Geometry check sheet. Reference: the model listing, model coordinates, mm. Face numbers are marked on the shaded views. A direction names the side the tool comes from. Round coordinates to 2 decimals unless told otherwise and drop trailing zeros. Write each loop counter-clockwise with the first axis right and the second up, starting at its lowest first coordinate (ties: lowest second). Pieces come first, ordered by that corner, then holes. Notation, with made-up numbers: (34.25, -5) -> (62.25, -5) arc R13 cw to (62.25, 18) -> close; hole circle Ø2 at (-36, 0.25). An arc over 180 degrees is marked (long way). Put each result on its own line as item: value. Start each with the question number.
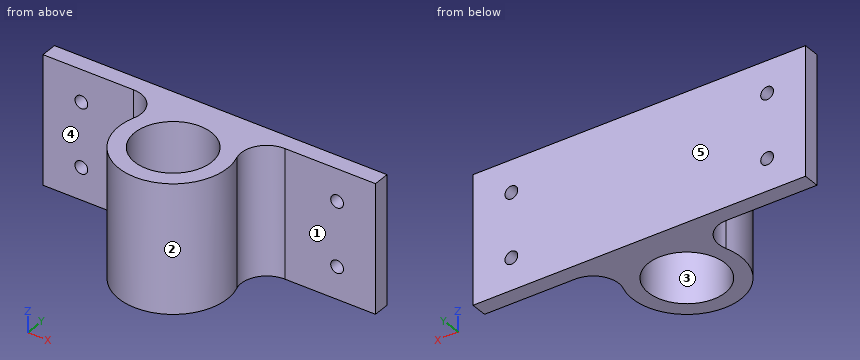
from build123d import *

# Parameters (mm, degrees)
SKETCH1_R           = 75
BOSS_EXTRUDE1_DEPTH = 250
CUT_EXTRUDE1_REACH  = 476.098
SKETCH2_R           = 12.5


with BuildPart() as part:
    # Sketch1 → Boss-Extrude1 (new body)
    with BuildSketch(Plane.XY):
        with BuildLine():
            Line((325, 132), (-325, 132))
            Line((-325, 132), (-325, 100))
            Line((-325, 100), (-147.770091697, 100))
            ThreePointArc((-147.770091697, 100), (-107.142009959, 79.143763902), (-100.407882819, 33.974358974))
            ThreePointArc((-100.407882819, 33.974358974), (0, -106), (100.407882819, 33.974358974))
            ThreePointArc((100.407882819, 33.974358974), (107.142009959, 79.143763902), (147.770091697, 100))
            Line((147.770091697, 100), (325, 100))
            Line((325, 100), (325, 132))
        make_face()
        Circle(SKETCH1_R, mode=Mode.SUBTRACT)
    extrude(amount=BOSS_EXTRUDE1_DEPTH)

    # Sketch2 → Cut-Extrude1 (cut, up to next)
    with BuildSketch(Plane(origin=(0, 132, 0), x_dir=(1, 0, 0), z_dir=(0, 1, 0)), mode=Mode.PRIVATE) as cut_extrude1_sk1:
        with Locations(Location((-250, -62.5, 0), (0, 0, 270))):
            Circle(SKETCH2_R)
    cut_extrude1_tool1 = extrude(cut_extrude1_sk1.sketch, amount=-CUT_EXTRUDE1_REACH, mode=Mode.PRIVATE) & part.part
    # Sketch2 → Cut-Extrude1 (cut, up to next)
    with BuildSketch(Plane(origin=(0, 132, 0), x_dir=(1, 0, 0), z_dir=(0, 1, 0)), mode=Mode.PRIVATE) as cut_extrude1_sk2:
        with Locations(Location((-250, -187.5, 0), (0, 0, 270))):
            Circle(SKETCH2_R)
    cut_extrude1_tool2 = extrude(cut_extrude1_sk2.sketch, amount=-CUT_EXTRUDE1_REACH, mode=Mode.PRIVATE) & part.part
    # Sketch2 → Cut-Extrude1 (cut, up to next)
    with BuildSketch(Plane(origin=(0, 132, 0), x_dir=(1, 0, 0), z_dir=(0, 1, 0)), mode=Mode.PRIVATE) as cut_extrude1_sk3:
        with Locations(Location((250, -187.5, 0), (0, 0, 270))):
            Circle(SKETCH2_R)
    cut_extrude1_tool3 = extrude(cut_extrude1_sk3.sketch, amount=-CUT_EXTRUDE1_REACH, mode=Mode.PRIVATE) & part.part
    # Sketch2 → Cut-Extrude1 (cut, up to next)
    with BuildSketch(Plane(origin=(0, 132, 0), x_dir=(1, 0, 0), z_dir=(0, 1, 0)), mode=Mode.PRIVATE) as cut_extrude1_sk4:
        with Locations(Location((250, -62.5, 0), (0, 0, 270))):
            Circle(SKETCH2_R)
    cut_extrude1_tool4 = extrude(cut_extrude1_sk4.sketch, amount=-CUT_EXTRUDE1_REACH, mode=Mode.PRIVATE) & part.part
    add(cut_extrude1_tool1.solids().sort_by_distance((-250, 132, 62.5))[0], mode=Mode.SUBTRACT)
    add(cut_extrude1_tool2.solids().sort_by_distance((-250, 132, 187.5))[0], mode=Mode.SUBTRACT)
    add(cut_extrude1_tool3.solids().sort_by_distance((250, 132, 187.5))[0], mode=Mode.SUBTRACT)
    add(cut_extrude1_tool4.solids().sort_by_distance((250, 132, 62.5))[0], mode=Mode.SUBTRACT)


solid = part.part
(1) Sectioned sample at D-D (x = -250). Record the cut outline in (y, z), and give its area (3 significant figures).
(2) Sectioned sample at C-C (z = 187.5). Record the cut outline in (x, y).
(3) Mould release check, pull along Y, two halves, no side actions. Record for the marked faces 3, 4 and 5: +Y half, -Y half, draft (parallel to the pull), parting line (faces both ways), or undercut.
(4) Sectioned sample at A-A (x = 0). Record the cut outline in (y, z), and give its area (3 significant figures).
(5) Go/stop test with flat-tipped pins: pin 1 Ø1.5 at (x, y) = (68.5, -41.5) entering from -Z; pin 2 Ø8 at (x, z) = (41.5, 172) entering from -Y; pin 3 Ø10 at (y, z) = (37.5, 119.5) entering from -X; pin 4 Ø1 at (y, z) = (-11.5, 27) entering from -X. Record where each tip stops, or that it passes through.
(6) Sectioned sample at B-B (y = 0). Record the cut outline in (x, z), and give its area (3 significant figures).
(7) Material ranges on L1, parallel to X at y = 109, z = 62.5; L2, parallel to Y at x = 0, z = 90; L3, parallel to Y at x = 274, z = 186.5, recorded low to high. Write a range as from..to.
(8) Set-up check for the marked faces 1 and 2: record each of +Z, -Z, +X, -X, +Y, -Y from which the full face is reachable in a straight line by a thin tool's end or side.
Found:
1. outline: (100, 0) -> (132, 0) -> (132, 50) -> (100, 50) -> close; (100, 75) -> (132, 75) -> (132, 175) -> (100, 175) -> close; (100, 200) -> (132, 200) -> (132, 250) -> (100, 250) -> close
1. area: 6,400 mm2
2. outline: (-325, 100) -> (-262.5, 100) -> (-262.5, 132) -> (-325, 132) -> close; (-237.5, 100) -> (-147.77, 100) arc R50 cw to (-100.41, 33.97) arc R106 ccw (long way) to (100.41, 33.97) arc R50 cw to (147.77, 100) -> (237.5, 100) -> (237.5, 132) -> (-237.5, 132) -> close; (262.5, 100) -> (325, 100) -> (325, 132) -> (262.5, 132) -> close; hole circle Ø150 at (0, 0)
3. face 3: undercut
3. face 4: -Y half
3. face 5: +Y half
4. outline: (-106, 0) -> (-75, 0) -> (-75, 250) -> (-106, 250) -> close; (75, 0) -> (132, 0) -> (132, 250) -> (75, 250) -> close
4. area: 22,000 mm2
5. pin 1: z = 0
5. pin 2: y = -99.15
5. pin 3: x = -100.89
5. pin 4: x = -105.43
6. outline: (-106, 0) -> (-75, 0) -> (-75, 250) -> (-106, 250) -> close; (75, 0) -> (106, 0) -> (106, 250) -> (75, 250) -> close
6. area: 15,500 mm2
7. L1: -325..-262.5, -237.5..237.5, 262.5..325
7. L2: -106..-75, 75..132
7. L3: 100..132
8. face 1: +Z, -Z, +X, -Y
8. face 2: +Z, -Z
